```python
from build123d import *

# Parameters (mm, degrees)
BOSS_EXTRUDE1_DEPTH     = 80
CHAMFER1_SIZE           = 1
CHAMFER2_SIZE           = 4
SKETCH2_W               = 8
SKETCH2_H               = 5
BOSS_EXTRUDE2_DEPTH     = 80
SKETCH3_R               = 4
CUT_EXTRUDE1_DEPTH      = 7.5
CUT_EXTRUDE2_DEPTH      = 86.234969349
CUT_EXTRUDE2_DEPTH_BACK = 86.234969349
SKETCH4_R               = 3
CUT_EXTRUDE3_DEPTH      = 89.090862182
CUT_EXTRUDE3_DEPTH_BACK = 3
SKETCH5_R               = 1.5


with BuildPart() as part:
    # Sketch1 → Boss-Extrude1 (new body)
    with BuildSketch(Plane(origin=(0, 0, 0), x_dir=(1, 0, 0), z_dir=(0, 1, 0))):
        Polygon((0, 25), (0, 0), (-24, 0), (-24, 7.06470747), (-20.721166606, 11), (-13.511532016, 11), (-13.511532016, 17.5), (-10, 17.5), (-10, 25), (-7, 25), (-7, 28), (-3, 28), (-3, 25), align=None)
    extrude(amount=BOSS_EXTRUDE1_DEPTH)

    # Chamfer1
    chamfer1_edges = [part.edges().sort_by_distance(p)[0] for p in [
        (-13.511532016, 40, -17.5),
        (-10, 40, -17.5),
        (-7, 40, -28),
        (-3, 40, -28),
        (0, 40, -25),
    ]]
    chamfer(chamfer1_edges, length=CHAMFER1_SIZE)

    # Chamfer2
    chamfer2_edges = [part.edges().sort_by_distance(p)[0] for p in [
        (-24, 80, -3.532353735),
        (-24, 0, -3.532353735),
    ]]
    chamfer(chamfer2_edges, length=CHAMFER2_SIZE)

    # Sketch2 → Boss-Extrude2 (add)
    with BuildSketch(Plane(origin=(0, 80, 0), x_dir=(1, 0, 0), z_dir=(0, 1, 0))):
        with Locations((-12, -2.5)):
            Rectangle(SKETCH2_W, SKETCH2_H)
    extrude(amount=-BOSS_EXTRUDE2_DEPTH)

    # Sketch3 → Cut-Extrude1 (cut, symmetric)
    with BuildSketch(Plane(origin=(0, 0, -11), x_dir=(-1, 0, 0), z_dir=(0, 0, -1))):
        with Locations((13.511532016, 52.5)):
            Circle(SKETCH3_R)
        with Locations(Location((13.511532016, 27.5, 0), (0, 0, 90))):
            Circle(SKETCH3_R)
    extrude(amount=CUT_EXTRUDE1_DEPTH, both=True, mode=Mode.SUBTRACT)

    # Sketch4 → Cut-Extrude2 (cut, two sides: drawn at the far end of the back side and taken through both)
    with BuildSketch(Plane(origin=(0, 0, -11), x_dir=(-1, 0, 0), z_dir=(0, 0, -1)).offset(-CUT_EXTRUDE2_DEPTH_BACK)):
        with Locations((13.511532016, 52.5)):
            Circle(SKETCH4_R)
        with Locations(Location((13.511532016, 27.5, 0), (0, 0, 33.953684666))):
            Circle(SKETCH4_R)
    extrude(amount=CUT_EXTRUDE2_DEPTH + CUT_EXTRUDE2_DEPTH_BACK, mode=Mode.SUBTRACT)

    # Sketch5 → Cut-Extrude3 (cut, two sides: drawn at the far end of the back side and taken through both)
    with BuildSketch(Plane.XY.offset(-CUT_EXTRUDE3_DEPTH_BACK)):
        with Locations(Location((-19, 40, 0), (0, 0, 180))):
            Circle(SKETCH5_R)
    extrude(amount=CUT_EXTRUDE3_DEPTH + CUT_EXTRUDE3_DEPTH_BACK, mode=Mode.SUBTRACT)


solid = part.part
```
For this review, take the finished solid that the model builds, in its own axes (mm). A direction names the side the tool comes from. Coordinates: 2 decimals unless noted, no trailing zeros. Write each loop counter-clockwise with the first axis right and the second up, starting at its lowest first coordinate (ties: lowest second). Pieces come first, ordered by that corner, then holes.
(1) The part is to be moulded in two halves that separate along Y. For faces 1 (the face through (-9.515, 52.676, -9.438)), 2 (the face through (-10, 39, -22)), 3 (the face through (-8, 0, -8)), say which applies: +Y half, -Y half, draft (parallel to the pull), parting line (faces both ways), or undercut.
(2) Add section B-B on z = -1.5. Give the boundary of the cut face in (x, y).
(3) Wall thickness on probe 1 along Y at (x, z) = (-12.25, -12); probe 2 along X at (y, z) = (27.5, -1.5); probe 3 along Z at (x, y) = (-16.5, 25): over which ranges is each line inside the solid? List them lowest first.
(4) Add section D-D on y = 21. Give the boundary of the cut face in (x, z).
(5) For pin 1 Ø3 at (y, z) = (72.5, -14) entering from -X; pin 2 Ø9.5 at (x, y) = (-13.51, 52.5) entering from +Z; pin 3 Ø6 at (y, z) = (37, -12.5) entering from -X; pin 4 Ø0.6 at (x, y) = (-2.5, 26) entering from -Z, all flat-tipped, find the tip position at first contact; note any pin that passes through.
(6) Add section A-A on y = 52.5. Give the boundary of the cut face in (x, z), then the cut area to 3 significant figures.
(7) Add section C-C on z = -5. Give the boundary of the cut face in (x, y), then the cut area to 3 significant figures.
(8) Tool access review of faces 4 (the face through (-8, 41, 3)), 5 (the face through (-21, 39, 0)), 6 (the face through (-19, 40, -3)), 7 (the face through (-13.512, 12, -14)): name each direction out of +Z, -Z, +X, -X, +Y, -Y from which nothing blocks a thin tool from reaching the whole face with its end or side.
Answer sheet:
1. face 1: undercut
1. face 2: draft
1. face 3: -Y half
2. outline: (-24, 4) - (-20, 0) - (0, 0) - (0, 80) - (-20, 80) - (-24, 76) - close; hole circle Ø3 at (-19, 40); hole circle Ø6 at (-13.51, 27.5); hole circle Ø6 at (-13.51, 52.5)
3. probe 1: y = 0 to 23.7, 31.3 to 48.7, 56.3 to 80
3. probe 2: x = -24 to -16.51, -10.51 to 0
3. probe 3: z = -3.5 to 0
4. outline: (-24, -7.06) - (-20.72, -11) - (-13.51, -11) - (-13.51, -16.5) - (-12.51, -17.5) - (-11, -17.5) - (-10, -18.5) - (-10, -25) - (-7, -25) - (-7, -27) - (-6, -28) - (-4, -28) - (-3, -27) - (-3, -25) - (-1, -25) - (0, -24) - (0, 0) - (-8, 0) - (-8, 5) - (-16, 5) - (-16, 0) - (-24, 0) - close
5. pin 1: stops at x = -13.51
5. pin 2: stops at z = 5
5. pin 3: stops at x = -21.97
5. pin 4: stops at z = -25
6. outline: (-24, -7.06) - (-20.72, -11) - (-17.51, -11) - (-17.51, -3.5) - (-16.51, -3.5) - (-16.51, 0) - (-24, 0) - close; (-10.51, -3.5) - (-9.51, -3.5) - (-9.51, -18.5) - (-10, -18.5) - (-10, -25) - (-7, -25) - (-7, -27) - (-6, -28) - (-4, -28) - (-3, -27) - (-3, -25) - (-1, -25) - (0, -24) - (0, 0) - (-8, 0) - (-8, 5) - (-10.51, 5) - close
6. area: 336 mm2
7. outline: (-24, 4) - (-20, 0) - (0, 0) - (0, 80) - (-20, 80) - (-24, 76) - close; hole circle Ø8 at (-13.51, 27.5); hole circle Ø8 at (-13.51, 52.5)
7. area: 1,800 mm2
8. face 4: +Z, +X, +Y, -Y
8. face 5: +Z, -X, +Y, -Y
8. face 6: +Z
8. face 7: -Z, -X, +Y, -Y
